Input: dimensioned drawing with shaded views. Units: mm. Origin: part minimum x, y, z. Round coordinates to 2 decimals unless told otherwise and drop trailing zeros. Loops run counter-clockwise (first coordinate to the right, second up) from the corner with the lowest first, then second, coordinate; pieces in that order, holes last.
Item 1: Section query A-A on y = 44. Return loops of the section in (x, z), then the cut area to 3 significant figures.
Item 2: Pull-direction query (Z, two-part tool) for the marked faces 1, 2, 3 and 4; classes: released by +Z, released by -Z, zero draft, split by the parting line, or undercut.
Item 3: Section query B-B on y = 8.5. Return loops of the section in (x, z).
Item 4: Section query C-C on x = 413. Return loops of the section in (y, z), then the cut area to 3 significant figures.
Item 5: Section query D-D on z = 330.5. Return loops of the section in (x, y), then the cut area to 3 significant figures.
Item 6: Ray query, L1, parallel to X at y = 16, z = 460; L2, parallel to Z at x = 459, y = 32; L3, parallel to X at y = 48, z = 345. Return the intervals inside material, ascending.
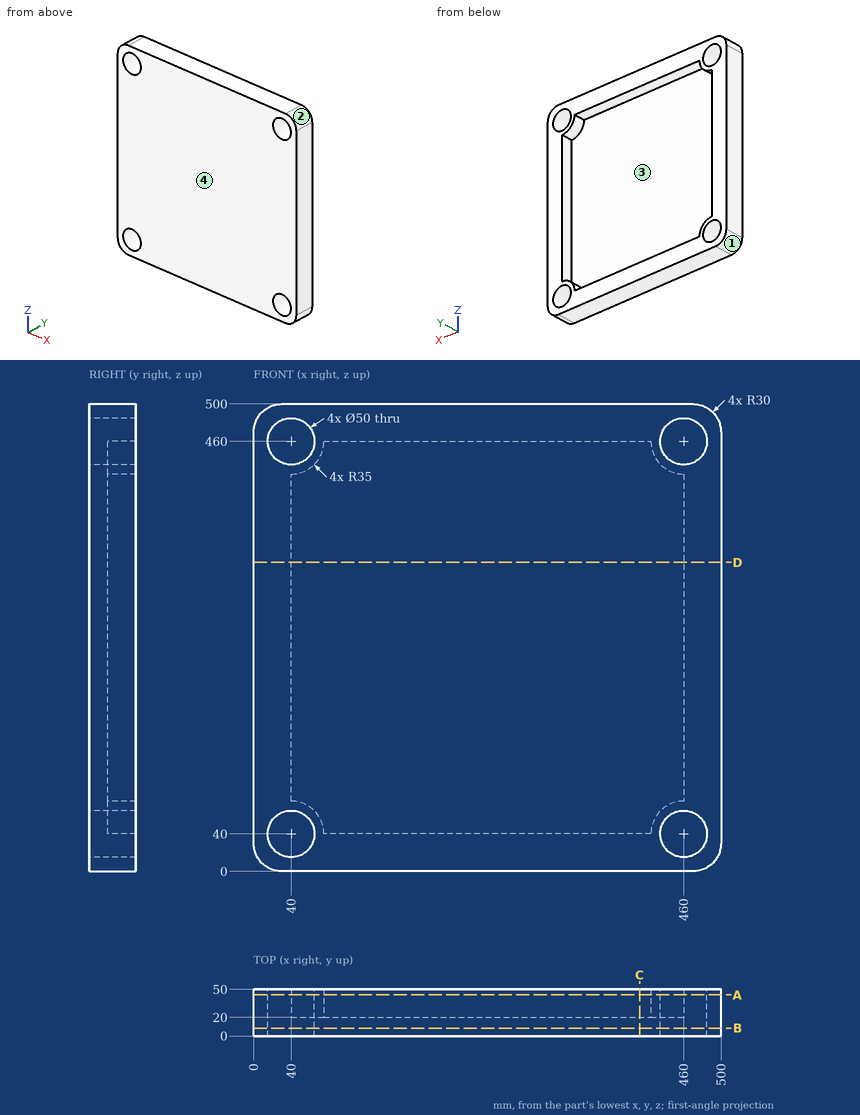
Data:
1. outline: (0, 30) arc R30 ccw to (30, 0) - (470, 0) arc R30 ccw to (500, 30) - (500, 470) arc R30 ccw to (470, 500) - (30, 500) arc R30 ccw to (0, 470) - close; hole circle Ø50 at (40, 40); hole circle Ø50 at (40, 460); hole (40, 75) arc R35 cw to (75, 40) - (425, 40) arc R35 cw to (460, 75) - (460, 425) arc R35 cw to (425, 460) - (75, 460) arc R35 cw to (40, 425) - close; hole circle Ø50 at (460, 40); hole circle Ø50 at (460, 460)
1. area: 68,800 mm2
2. face 1: released by -Z
2. face 2: released by +Z
2. face 3: undercut
2. face 4: zero draft
3. outline: (0, 30) arc R30 ccw to (30, 0) - (470, 0) arc R30 ccw to (500, 30) - (500, 470) arc R30 ccw to (470, 500) - (30, 500) arc R30 ccw to (0, 470) - close; hole circle Ø50 at (40, 40); hole circle Ø50 at (40, 460); hole circle Ø50 at (460, 40); hole circle Ø50 at (460, 460)
4. outline: (0, 0) - (50, 0) - (50, 40) - (20, 40) - (20, 460) - (50, 460) - (50, 500) - (0, 500) - close
4. area: 12,400 mm2
5. outline: (0, 0) - (500, 0) - (500, 50) - (460, 50) - (460, 20) - (40, 20) - (40, 50) - (0, 50) - close
5. area: 12,400 mm2
6. L1: x = 0 to 15, 65 to 435, 485 to 500
6. L2: z = 0 to 15.02, 64.98 to 74.99, 425.01 to 435.02, 484.98 to 500
6. L3: x = 0 to 40, 460 to 500
